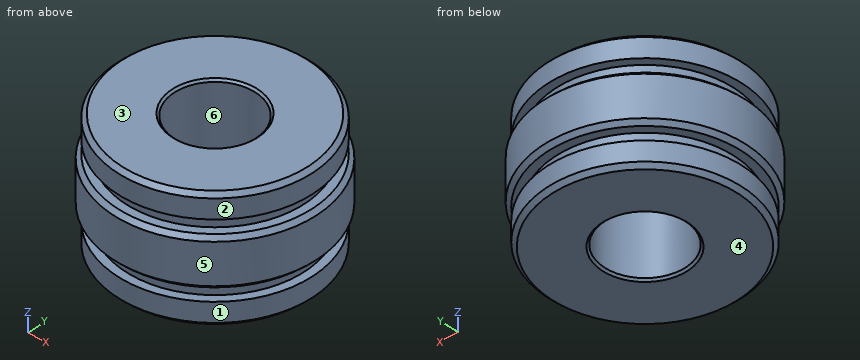
from build123d import *

# Parameters (mm, degrees)
SKETCH1_R           = 50
SKETCH1_R_2         = 20
BOSS_EXTRUDE1_DEPTH = 60
CUT_EXTRUDE1_START  = -42
SKETCH2_R           = 50
SKETCH2_R_2         = 44
CUT_EXTRUDE1_DEPTH  = 6.5
CUT_EXTRUDE2_START  = 11.5
SKETCH3_R           = 50
SKETCH3_R_2         = 44
CUT_EXTRUDE2_DEPTH  = 6.5
CUT_EXTRUDE3_START  = -12
SKETCH5_R           = 50
SKETCH5_R_2         = 48
CUT_EXTRUDE3_DEPTH  = 12
SKETCH6_R           = 50
SKETCH6_R_2         = 48
CUT_EXTRUDE4_DEPTH  = 12
CHAMFER1_SIZE       = 2
CHAMFER2_SIZE       = 1
CHAMFER3_SIZE       = 2


with BuildPart() as part:
    # Sketch1 → Boss-Extrude1 (new body)
    with BuildSketch(Plane.XY):
        Circle(SKETCH1_R)
        Circle(SKETCH1_R_2, mode=Mode.SUBTRACT)
    extrude(amount=BOSS_EXTRUDE1_DEPTH)

    # Sketch2 → Cut-Extrude1 (cut)
    with BuildSketch(Plane(origin=(0, 0, 0), x_dir=(-1, 0, 0), z_dir=(0, 0, -1)).offset(CUT_EXTRUDE1_START)):
        Circle(SKETCH2_R)
        Circle(SKETCH2_R_2, mode=Mode.SUBTRACT)
    extrude(amount=-CUT_EXTRUDE1_DEPTH, mode=Mode.SUBTRACT)

    # Sketch3 → Cut-Extrude2 (cut)
    with BuildSketch(Plane.XY.offset(CUT_EXTRUDE2_START)):
        Circle(SKETCH3_R)
        with Locations(Location((0, 0, 0), (0, 0, 180))):
            Circle(SKETCH3_R_2, mode=Mode.SUBTRACT)
    extrude(amount=CUT_EXTRUDE2_DEPTH, mode=Mode.SUBTRACT)

    # Sketch5 → Cut-Extrude3 (cut)
    with BuildSketch(Plane.XY.offset(60).offset(CUT_EXTRUDE3_START)):
        Circle(SKETCH5_R)
        Circle(SKETCH5_R_2, mode=Mode.SUBTRACT)
    extrude(amount=CUT_EXTRUDE3_DEPTH, mode=Mode.SUBTRACT)

    # Sketch6 → Cut-Extrude4 (cut)
    with BuildSketch(Plane(origin=(0, 0, 0), x_dir=(-1, 0, 0), z_dir=(0, 0, -1))):
        Circle(SKETCH6_R)
        with Locations(Location((0, 0, 0), (0, 0, 180))):
            Circle(SKETCH6_R_2, mode=Mode.SUBTRACT)
    extrude(amount=-CUT_EXTRUDE4_DEPTH, mode=Mode.SUBTRACT)

    # Chamfer1
    chamfer1_edges = [part.edges().sort_by_distance(p)[0] for p in [
        (-48, 0, 60),
        (-48, 0, 0),
    ]]
    chamfer(chamfer1_edges, length=CHAMFER1_SIZE)

    # Chamfer2
    chamfer2_edges = [part.edges().sort_by_distance(p)[0] for p in [
        (-20, 0, 0),
        (-20, 0, 60),
    ]]
    chamfer(chamfer2_edges, length=CHAMFER2_SIZE)

    # Chamfer3
    chamfer3_edges = [part.edges().sort_by_distance(p)[0] for p in [
        (-50, 0, 42),
        (-50, 0, 18),
    ]]
    chamfer(chamfer3_edges, length=CHAMFER3_SIZE)


solid = part.part
Model file for the job. Use its own axes, mm. Face numbers are marked on the shaded views. A direction names the side the tool comes from. Give positions to 0.01 mm unless a question says otherwise; leave off trailing zeros. Order: outer loops, then holes, each group sorted by start corner. A loop starts at its lowest first (then second) coordinate and runs counter-clockwise, first axis right, second up. Notation, with made-up numbers: (33.25, 30) - (59.25, 30) arc R23 ccw to (59.25, 40) - close; hole circle Ø10 at (-16.75, 26). An arc over 180 degrees is marked (long way). One line per item, written item: value.
Item 1: Wall check: line 1 (Y direction, x = 0, z = 22.5); line 2 (Y direction, x = -10, z = 55.5); line 3 (X direction, y = -1.5, z = 15). Give the ranges that are in metal, low to high.
Response values:
line 1: -50 to -20, 20 to 50
line 2: -46.95 to -17.32, 17.32 to 46.95
line 3: -43.97 to -19.94, 19.94 to 43.97
Item 2: Slice it at A-A (z = 7). List the corners of the cut face in (x, y).
Response values:
outline: circle Ø96 at (0, 0); hole circle Ø40 at (0, 0)
Item 3: Tool access for the marked faces 1, 2 and 3: list every direction of +Z, -Z, +X, -X, +Y, -Y with a clear straight run to the whole face (end or side of a thin tool).
Response values:
face 1: -Z
face 2: +Z
face 3: +Z, +X, -X, +Y, -Y
Item 4: Two-plate mould, pull along Y, no slides. Class the marked faces 4, 5 and 6: released by +Y, released by -Y, zero draft, split by the parting line, or undercut.
Response values:
face 4: zero draft
face 5: split by the parting line
face 6: undercut
Item 5: Slice it at B-B (z = 14.5). List the corners of the cut face in (x, y).
Response values:
outline: circle Ø88 at (0, 0); hole circle Ø40 at (0, 0)
Item 6: Pin check, flat tips, straight feed: pin 1 Ø8 at (x, z) = (20.5, 9) entering from +Y; pin 2 Ø2 at (y, z) = (31.5, 47) entering from +X; pin 3 Ø8 at (x, z) = (-5, 46.5) entering from -Y. Stop position of each tip, or through.
Response values:
pin 1: y = 45.07
pin 2: x = 31.71
pin 3: y = -47.98
